from build123d import *

# Parameters (mm, degrees)
SKETCH1_W           = 141
SKETCH1_H           = 60
BOSS_EXTRUDE1_DEPTH = 4
M4_TAPPED_HOLE1_D   = 3.3


with BuildPart() as part:
    # Sketch1 → Boss-Extrude1 (new body)
    with BuildSketch(Plane(origin=(0, 0, 0), x_dir=(1, 0, 0), z_dir=(0, 1, 0))):
        Rectangle(SKETCH1_W, SKETCH1_H)
    extrude(amount=BOSS_EXTRUDE1_DEPTH)

    # M4 Tapped Hole1 (through all)
    with Locations(Plane(origin=(0, 4, 0), x_dir=(1, 0, 0), z_dir=(0, 1, 0))):
        with Locations((-40, 0), (0, 0), (40, 0)):
            Hole(M4_TAPPED_HOLE1_D / 2)


solid = part.part
Source: CAD feature listing. Evaluate the final solid. Frame: model axes, mm. Coordinates: 2 decimals unless noted, no trailing zeros. Order: outer loops, then holes, each group sorted by start corner. A loop starts at its lowest first (then second) coordinate and runs counter-clockwise, first axis right, second up. Notation, with made-up numbers: M 71.25,4.5 L 93.25,4.5 A25 ccw 93.25,19.5 Z; hole C -25,22 d7. An arc over 180 degrees is marked long. Write each question's results on one line, items separated by ' | '. Start each with the question number.
Item 1: Cut plane B-B (z = 0). Return loops of the section in (x, y), and give its area (3 significant figures).
Item 2: Line query: probe 1 along Z at (x, y) = (40, 2.45); probe 2 along X at (y, z) = (2.9, -0.5); probe 3 along X at (y, z) = (2.15, -1). Output: solid intervals per line, ascending.
Item 3: Draft query along Z for faces 1 (the face through (-1, 2, -30)), 2 (the face through (41.65, 1.97, -0.07)), 3 (the face through (-70.5, 2, 0)). Return one class per face: pulls with the +Z half, pulls with the -Z half, needs draft (parallel to the pull), parting line crosses it, or undercut.
Item 4: Cut plane A-A (x = -40). Return loops of the section in (y, z).
Checked values:
1) outline: M -70.5,0 L -41.65,0 L -41.65,4 L -70.5,4 Z; M -38.35,0 L -1.65,0 L -1.65,4 L -38.35,4 Z; M 1.65,0 L 38.35,0 L 38.35,4 L 1.65,4 Z; M 41.65,0 L 70.5,0 L 70.5,4 L 41.65,4 Z | area: 524 mm2
2) probe 1: z = -30 to -1.65, 1.65 to 30 | probe 2: x = -70.5 to -41.57, -38.43 to -1.57, 1.57 to 38.43, 41.57 to 70.5 | probe 3: x = -70.5 to -41.31, -38.69 to -1.31, 1.31 to 38.69, 41.31 to 70.5
3) face 1: pulls with the -Z half | face 2: undercut | face 3: needs draft
4) outline: M 0,-30 L 4,-30 L 4,-1.65 L 0,-1.65 Z; M 0,1.65 L 4,1.65 L 4,30 L 0,30 Z
